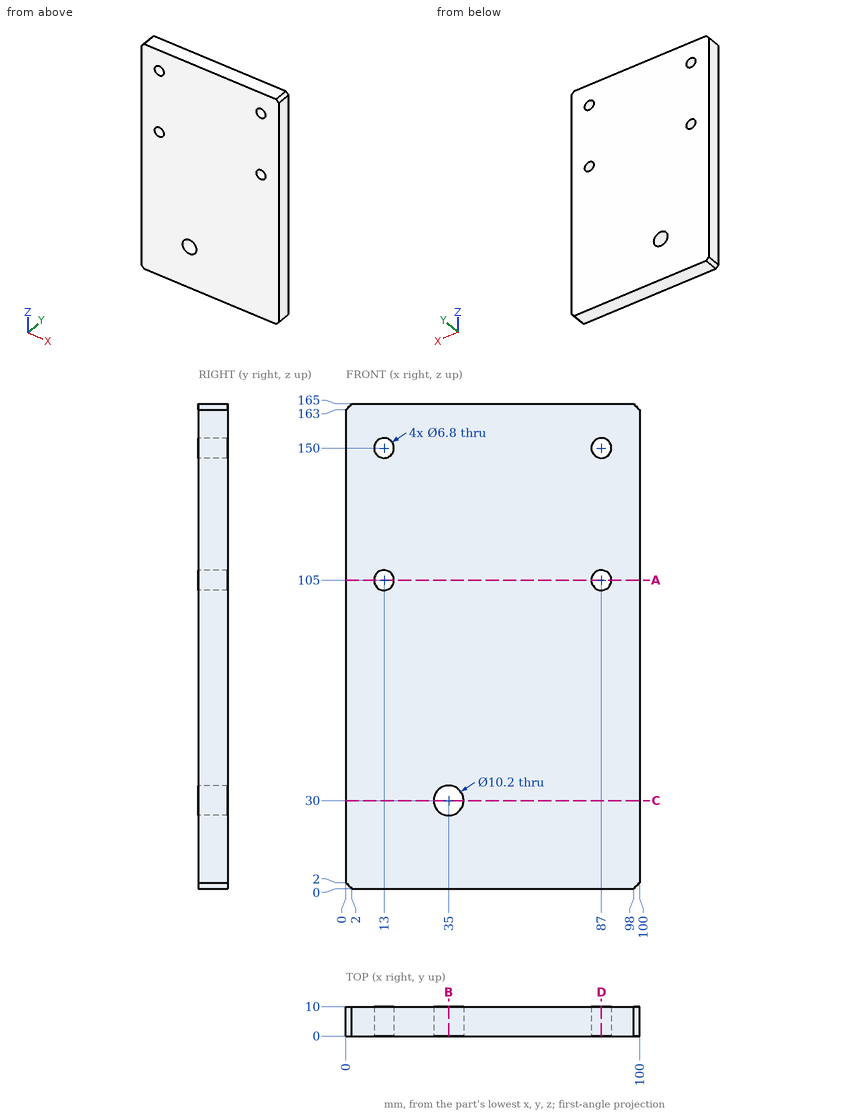
The figure shows three views and two pictorial views of one solid part (mm, origin at its lowest corner). Answer the questions. Coordinates: 2 decimals unless noted, no trailing zeros. Order: outer loops, then holes, each group sorted by start corner. A loop starts at its lowest first (then second) coordinate and runs counter-clockwise, first axis right, second up. Notation, with made-up numbers: M -26,4 L -9,4 A24 cw -9,29 Z; hole C 22.5,42.5 d6. An arc over 180 degrees is marked long. Use CSV: the item, a comma, the result in double quotes.
1) Section A-A on z = 105 is taken. Write down the section's boundary in (x, y).
Worked out:
outline,"M 0,0 L 9.6,0 L 9.6,10 L 0,10 Z; M 16.4,0 L 83.6,0 L 83.6,10 L 16.4,10 Z; M 90.4,0 L 100,0 L 100,10 L 90.4,10 Z"
2) Section C-C on z = 30 is taken. Write down the section's boundary in (x, y), plus the area to 3 significant figures.
Worked out:
outline,"M 0,0 L 29.9,0 L 29.9,10 L 0,10 Z; M 40.1,0 L 100,0 L 100,10 L 40.1,10 Z"
area,"898 mm^2"
3) Section B-B on x = 35 is taken. Write down the section's boundary in (y, z), plus the area to 3 significant figures.
Worked out:
outline,"M 0,0 L 10,0 L 10,24.9 L 0,24.9 Z; M 0,35.1 L 10,35.1 L 10,165 L 0,165 Z"
area,"1,550 mm^2"
4) Section D-D on x = 87 is taken. Write down the section's boundary in (y, z), plus the area to 3 significant figures.
Worked out:
outline,"M 0,0 L 10,0 L 10,101.6 L 0,101.6 Z; M 0,108.4 L 10,108.4 L 10,146.6 L 0,146.6 Z; M 0,153.4 L 10,153.4 L 10,165 L 0,165 Z"
area,"1,510 mm^2"
5) Consider line 1 (X direction, y = 2.25, z = 105); line 2 (Z direction, x = 13, y = 6); line 3 (X direction, y = 4, z = 102). Determine where each line is inside the solid, lowest interval first. Write a range as [from, to].
Worked out:
line 1,"x = [0, 9.6], [16.4, 83.6], [90.4, 100]"
line 2,"z = [0, 101.6], [108.4, 146.6], [153.4, 165]"
line 3,"x = [0, 11.4], [14.6, 85.4], [88.6, 100]"
6) Flat-ended cylindrical pins translate along their axes: pin 1 Ø13.5 at (x, z) = (35, 30) entering from +Y; pin 2 Ø5.5 at (x, z) = (13, 105) entering from -Y. Find the tip coordinate at first contact, or state that the pin passes through.
Worked out:
pin 1,"stops at y = 10"
pin 2,"passes through"
